Answer from the drawing. Dimensions are ordinates in mm from the lowest x, y and z of the part. Round coordinates to 2 decimals unless told otherwise and drop trailing zeros. Order: outer loops, then holes, each group sorted by start corner. A loop starts at its lowest first (then second) coordinate and runs counter-clockwise, first axis right, second up. Notation, with made-up numbers: M -5,78 L 45,78 A18 ccw 45,98 Z; hole C 7.5,-4 d3. An arc over 180 degrees is marked long. Answer as a JSON object with one key per item and string values. Group by question number.
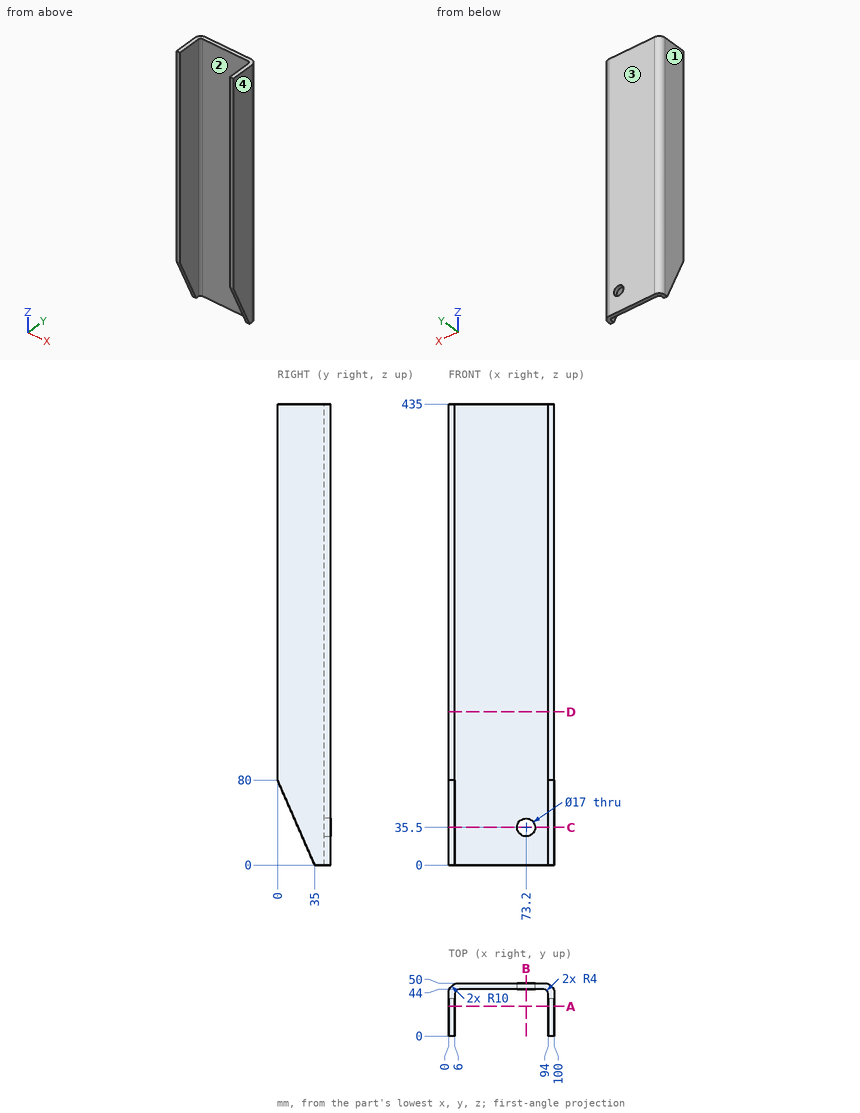
Item 1: Each of these flat-tipped pins is pushed along its axis until it touches: pin 1 (5 mm diameter, centred on y = 43, z = 245, fed in from +X); pin 2 (6 mm diameter, centred on x = 47, z = 191, fed in from -Y); pin 3 (15.5 mm diameter, centred on x = 73.2, z = 35.5, fed in from +Y). Where does it stop, or does it pass through?
Item 2: Find section B-B (x = 73.2). Give the vertices of the cut face in (y, z), and give its area (3 significant figures).
Item 3: Consider L1, parallel to X at y = 17, z = 128; L2, parallel to Z at x = 73, y = 46; L3, parallel to Y at x = 59, z = 185. Determine where each line is inside the solid, lowest interval first.
Item 4: Find section A-A (y = 28). Give the vertices of the cut face in (x, z).
Item 5: Find section C-C (z = 35.5). Give the vertices of the cut face in (x, y).
Item 6: Find section D-D (z = 144.5). Give the vertices of the cut face in (x, y).
Item 7: The mould has two halves that part along X. Classify the marked faces 1, 2, 3 and 4: +X half, -X half, draft (parallel to the pull), parting line (faces both ways), or undercut.
Responses:
{
 "1": {"pin 1": "stops at x = 99.99", "pin 2": "stops at y = 44", "pin 3": "passes through"},
 "2": {"outline": "M 44,0 L 50,0 L 50,27 L 44,27 Z; M 44,44 L 50,44 L 50,435 L 44,435 Z", "area": "2,510 mm^2"},
 "3": {"L1": "x = 0 to 6, 94 to 100", "L2": "z = 0 to 27, 44 to 435", "L3": "y = 44 to 50"},
 "4": {"outline": "M 0,16 L 6,16 L 6,435 L 0,435 Z; M 94,16 L 100,16 L 100,435 L 94,435 Z"},
 "5": {"outline": "M 0,19.47 L 6,19.47 L 6,40 A4 cw 10,44 L 64.7,44 L 64.7,50 L 10,50 A10 ccw 0,40 Z; M 81.7,44 L 90,44 A4 cw 94,40 L 94,19.47 L 100,19.47 L 100,40 A10 ccw 90,50 L 81.7,50 Z"},
 "6": {"outline": "M 0,0 L 6,0 L 6,40 A4 cw 10,44 L 90,44 A4 cw 94,40 L 94,0 L 100,0 L 100,40 A10 ccw 90,50 L 10,50 A10 ccw 0,40 Z"},
 "7": {"face 1": "-X half", "face 2": "undercut", "face 3": "draft", "face 4": "+X half"}
}
